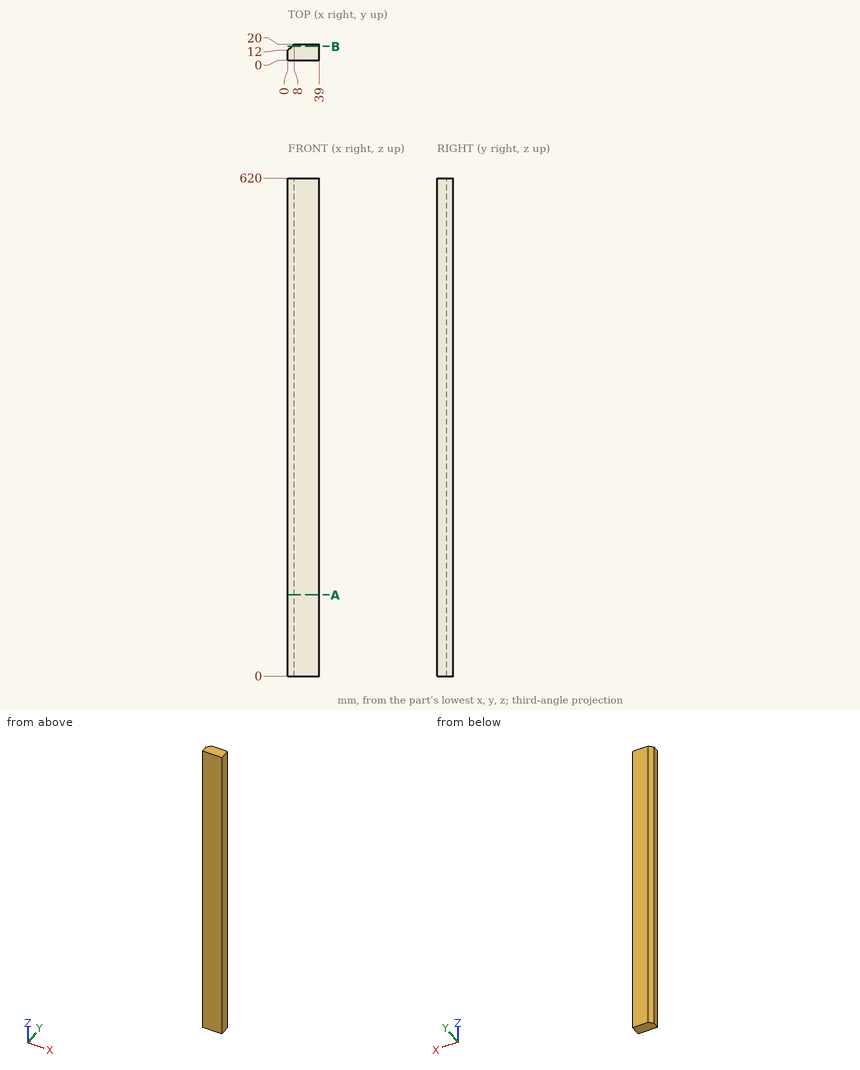
Job drawing, mm, ordinate dimensions from the low corner. One solid piece. Round coordinates to 2 decimals unless told otherwise and drop trailing zeros. Loops run counter-clockwise (first coordinate to the right, second up) from the corner with the lowest first, then second, coordinate; pieces in that order, holes last. Notation, with made-up numbers: (41, 73.25) -> (53, 73.25) arc R18 ccw to (53, 92.25) -> close; hole circle Ø4 at (-0.5, 27.5). An arc over 180 degrees is marked (long way). One line per item, written item: value. Start each with the question number.
Q1. Probe line 1 along X through (y, z) = (17.25, 386.5); line 2 along X through (y, z) = (15.75, 228). List the from-to ranges inside material, lowest first.
Q2. Cut at A-A on z = 101. List the corners of the cut face in (x, y), plus the area to 3 significant figures.
Q3. Cut at B-B on y = 17. List the corners of the cut face in (x, z), plus the area to 3 significant figures.
Computed:
1. line 1: 5.25 to 39
1. line 2: 3.75 to 39
2. outline: (0, 0) -> (39, 0) -> (39, 20) -> (8, 20) -> (0, 12) -> close
2. area: 748 mm²
3. outline: (5, 0) -> (39, 0) -> (39, 620) -> (5, 620) -> close
3. area: 21,100 mm²
